Work out the finished part from the listing and answer in its coordinate system (mm). A direction names the side the tool comes from. Round coordinates to 2 decimals unless told otherwise and drop trailing zeros. Order: outer loops, then holes, each group sorted by start corner. A loop starts at its lowest first (then second) coordinate and runs counter-clockwise, first axis right, second up. Notation, with made-up numbers: M -35.75,-0.5 L 7.25,-0.5 A4 cw 7.25,3.5 Z; hole C 0.5,76 d9. An arc over 180 degrees is marked long. Return JSON: item names as keys, results as strings.
from build123d import *

# Parameters (mm, degrees)
SKETCH1_W              = 70
SKETCH1_H              = 70
BOSS_EXTRUDE1_DEPTH    = 65
SKETCH2_R              = 12.5
BOSS_EXTRUDE2_DEPTH    = 10
M16_TAPPED_HOLE1_D     = 14
M16_TAPPED_HOLE1_DEPTH = 42
M16_TAPPED_HOLE1_TIP   = 4.206024333


with BuildPart() as part:
    # Sketch1 → Boss-Extrude1 (new body)
    with BuildSketch(Plane.XY):
        Rectangle(SKETCH1_W, SKETCH1_H)
    extrude(amount=BOSS_EXTRUDE1_DEPTH)

    # Sketch2 → Boss-Extrude2 (add)
    with BuildSketch(Plane.XY.offset(65)):
        Circle(SKETCH2_R)
    extrude(amount=BOSS_EXTRUDE2_DEPTH)

    # M16 Tapped Hole1
    with Locations(Plane.XY.offset(75)):
        with Locations((0, 0)):
            Hole(M16_TAPPED_HOLE1_D / 2, depth=M16_TAPPED_HOLE1_DEPTH)
            with Locations((0, 0, -(M16_TAPPED_HOLE1_DEPTH + M16_TAPPED_HOLE1_TIP / 2))):  # 118° drill point
                Cone(0, M16_TAPPED_HOLE1_D / 2, M16_TAPPED_HOLE1_TIP, mode=Mode.SUBTRACT)


solid = part.part
Item 1: Find section D-D (x = 9.5). Determine the outline of the cut face in (y, z), plus the area to 3 significant figures.
Output:
{"outline": "M -35,0 L 35,0 L 35,65 L 8.12,65 L 8.12,75 L -8.12,75 L -8.12,65 L -35,65 Z", "area": "4,710 mm^2"}
Item 2: Find section A-A (z = 37). Determine the outline of the cut face in (x, y), plus the area to 3 significant figures.
Output:
{"outline": "M -35,-35 L 35,-35 L 35,35 L -35,35 Z; hole C 0,0 d14", "area": "4,750 mm^2"}
Item 3: Find section B-B (x = -16.5). Determine the outline of the cut face in (y, z).
Output:
{"outline": "M -35,0 L 35,0 L 35,65 L -35,65 Z"}
Item 4: Consider line 1 along Y through (x, z) = (0, 62); line 2 along Z through (x, y) = (20, -12). Determine where each line is inside the solid, lowest interval first. Write a range as [from, to].
Output:
{"line 1": "y = [-35, -7], [7, 35]", "line 2": "z = [0, 65]"}
Item 5: The mould has two halves that part along Y. Classify faces 3 (the flat face through (0, 35, 32)), 4 (the cylindrical face through (-6.466, -2.681, 53.706)), 5 (the conical face through (-0.264, -1.187, 29.524)), 6 (the flat face through (0, 0, 0)): pulls with the +Y half, pulls with the -Y half, needs draft (parallel to the pull), parting line crosses it, or undercut.
Output:
{"face 3": "pulls with the +Y half", "face 4": "undercut", "face 5": "undercut", "face 6": "needs draft"}
Item 6: Which of the six approach directions +Z, -Z, +X, -X, +Y, -Y give full straight-line access (tool end or side, diameter ignored) to faces 1 (the cylindrical face through (11.923, 3.755, 69.93)), 2 (the flat face through (35, 0, 32))?
Output:
{"face 1": "+Z", "face 2": "+Z, -Z, +X, +Y, -Y"}
Item 7: This flat-tipped pin is pushed along its axis until it touches: pin 1 (3 mm diameter, centred on x = 2.5, y = -17.5, fed in from -Z). Where does it stop, or does it pass through?
Output:
{"pin 1": "stops at z = 0"}
